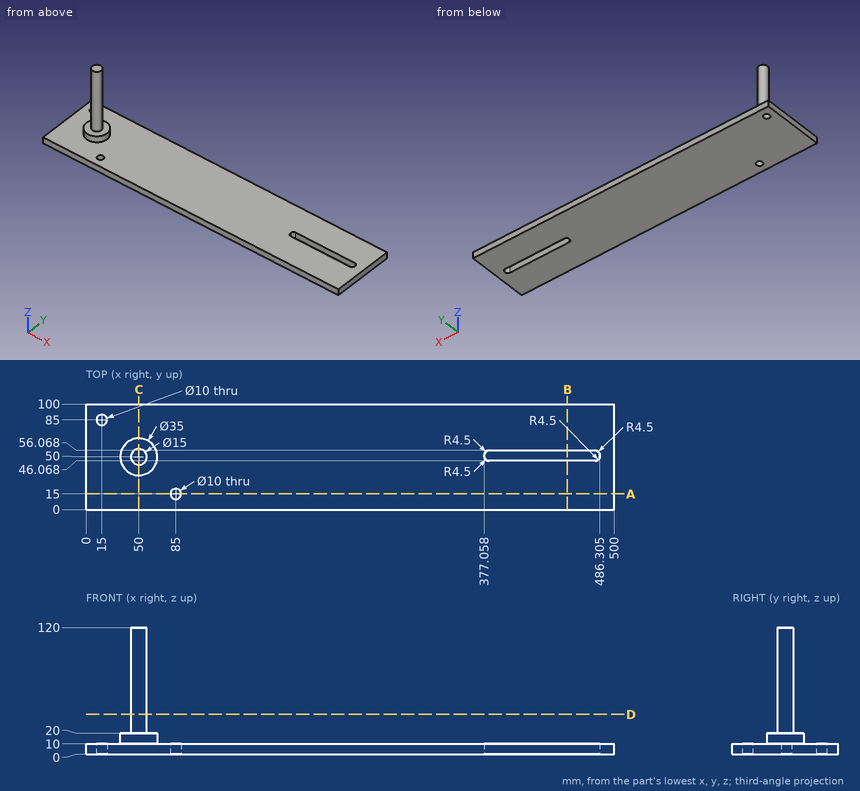
Input: dimensioned drawing with shaded views. Units: mm. Origin: part minimum x, y, z. Give positions to 0.01 mm unless a question says otherwise; leave off trailing zeros. Write each loop counter-clockwise with the first axis right and the second up, starting at its lowest first coordinate (ties: lowest second). Pieces come first, ordered by that corner, then holes. Notation, with made-up numbers: (-0.5, 62) - (47.5, 62) arc R20 cw to (47.5, 96) - close; hole circle Ø1 at (52, 40.25). An arc over 180 degrees is marked (long way). One line per item, written item: value. Start each with the question number.
Q1. First-contact query: pin 1 Ø2 at (x, y) = (436, 79) entering from +Z. Flat tip, straight axial feed; report the tip coordinate or a pass-through.
Q2. Material intervals for probe 1 along Y at (x, z) = (15, 4.25); probe 2 along Z at (x, y) = (346.5, 72.5); probe 3 along Y at (x, z) = (85, 5), sorted ascending. Write a range as from..to.
Q3. Section query D-D, the plane z = 38. Return the cut outline in (x, y), then the cut area to 3 significant figures.
Q4. Section query A-A, the plane y = 15. Return the cut outline in (x, z).
Q5. Section query B-B, the plane x = 455.5. Return the cut outline in (y, z), then the cut area to 3 significant figures.
Q6. Section query C-C, the plane x = 50. Return the cut outline in (y, z), then the cut area to 3 significant figures.
Answer:
1. pin 1: stops at z = 10
2. probe 1: y = 0..80, 90..100
2. probe 2: z = 0..10
2. probe 3: y = 0..10, 20..100
3. outline: circle Ø15 at (50, 50)
3. area: 177 mm2
4. outline: (0, 0) - (80, 0) - (80, 10) - (0, 10) - close; (90, 0) - (500, 0) - (500, 10) - (90, 10) - close
5. outline: (0, 0) - (46.07, 0) - (46.07, 10) - (0, 10) - close; (56.07, 0) - (100, 0) - (100, 10) - (56.07, 10) - close
5. area: 900 mm2
6. outline: (0, 0) - (100, 0) - (100, 10) - (67.5, 10) - (67.5, 20) - (57.5, 20) - (57.5, 120) - (42.5, 120) - (42.5, 20) - (32.5, 20) - (32.5, 10) - (0, 10) - close
6. area: 2,850 mm2
